The model under review builds one solid part; all positions refer to its coordinate system, in mm. A direction names the side the tool comes from. Round coordinates to 2 decimals unless told otherwise and drop trailing zeros. Loops run counter-clockwise (first coordinate to the right, second up) from the corner with the lowest first, then second, coordinate; pieces in that order, holes last. Notation, with made-up numbers: (-17.5, 56) - (29.5, 56) arc R33 ccw to (29.5, 89) - close; hole circle Ø2 at (-30.75, 75). An arc over 180 degrees is marked (long way). Answer as CSV lines item,"result".
from build123d import *

# Parameters (mm, degrees)
SKETCH_1_R          = 15
EXTRUDE_1_DEPTH     = 2.8
EXTRUDE_2_DEPTH     = 5.4
SKETCH_3_R          = 13.05
EXTRUDE_3_DEPTH     = 7
SKETCH_4_R          = 9.5
CUT_EXTRUDE_1_DEPTH = 13


with BuildPart() as part:
    # 草图1 → 凸台-拉伸1 (new body)
    with BuildSketch(Plane.XY):
        Circle(SKETCH_1_R)
    extrude(amount=EXTRUDE_1_DEPTH)

    # 草图2 → 凸台-拉伸2 (add)
    with BuildSketch(Plane(origin=(0, 0, 0), x_dir=(-1, 0, 0), z_dir=(0, 0, -1))):
        Polygon((6.062177826, -10.5), (12.124355653, 0), (6.062177826, 10.5), (-6.062177826, 10.5), (-12.124355653, 0), (-6.062177826, -10.5), align=None)
    extrude(amount=EXTRUDE_2_DEPTH)

    # 草图3 → 凸台-拉伸3 (add)
    with BuildSketch(Plane.XY.offset(2.8)):
        Circle(SKETCH_3_R)
    extrude(amount=EXTRUDE_3_DEPTH)

    # 草图4 → 切除-拉伸1 (cut)
    with BuildSketch(Plane.XY.offset(9.8)):
        Circle(SKETCH_4_R)
    extrude(amount=-CUT_EXTRUDE_1_DEPTH, mode=Mode.SUBTRACT)


solid = part.part
1. Clearance check with flat-ended pins moving along their axes: pin 1 (2.5 mm diameter, centred on x = -2, z = -3.5, fed in from -Y); pin 2 (6 mm diameter, centred on y = 6.5, z = 0.5, fed in from +X); pin 3 (3 mm diameter, centred on y = 10.5, z = -0.5, fed in from -X). State where each tip first meets the part, or that it passes through.
Numbers:
pin 1,"stops at y = -10.5"
pin 2,"stops at x = 14.59"
pin 3,"stops at x = -11.94"
2. Take a section at D-D (z = -4.25). State the section outline as (x, y) points.
Numbers:
outline,"(-12.12, 0) - (-6.06, -10.5) - (6.06, -10.5) - (12.12, 0) - (6.06, 10.5) - (-6.06, 10.5) - close"
3. Tool access review of faces 1 (the face through (-9.136, 5.176, -2.662)), 2 (the face through (0, -11, 0)), 3 (the face through (-1.2, -13.3, 2.8)): name each direction out of +Z, -Z, +X, -X, +Y, -Y from which nothing blocks a thin tool from reaching the whole face with its end or side.
Numbers:
face 1,"-Z, -X, +Y"
face 2,"-Z"
face 3,"+Z"
4. Take a section at C-C (y = 12). State the section outline as (x, z) points, plus the area to 3 significant figures.
Numbers:
outline,"(-9, 0) - (9, 0) - (9, 2.8) - (5.13, 2.8) - (5.13, 9.8) - (-5.13, 9.8) - (-5.13, 2.8) - (-9, 2.8) - close"
area,"122 mm²"
5. Take a section at A-A (z = -2.5). State the section outline as (x, y) points, plus the area to 3 significant figures.
Numbers:
outline,"(-12.12, 0) - (-6.06, -10.5) - (6.06, -10.5) - (12.12, 0) - (6.06, 10.5) - (-6.06, 10.5) - close; hole circle Ø19 at (0, 0)"
area,"98.4 mm²"
6. Wall thickness on probe 1 along Y at (x, z) = (0.25, -1); probe 2 along Y at (x, z) = (0, 1); probe 3 along X at (y, z) = (7.5, -3): over which ranges is each line inside the solid? List them lowest first.
Numbers:
probe 1,"y = -10.5 to -9.5, 9.5 to 10.5"
probe 2,"y = -15 to -9.5, 9.5 to 15"
probe 3,"x = -7.79 to -5.83, 5.83 to 7.79"
7. Draft analysis for pull direction X (two halves, no side actions). For faces 4 (the face through (4.38, -8.43, 3.39)), 5 (the face through (0, 0, -3.2)), 6 (the face through (-9.051, -5.324, -2.662)), 7 (the face through (1, -10, 9.8)), state which applies: +X half, -X half, draft (parallel to the pull), parting line (faces both ways), or undercut.
Numbers:
face 4,"undercut"
face 5,"undercut"
face 6,"-X half"
face 7,"draft"
8. Take a section at B-B (x = 0). State the section outline as (y, z) points, plus the area to 3 significant figures.
Numbers:
outline,"(-15, 0) - (-10.5, 0) - (-10.5, -5.4) - (10.5, -5.4) - (10.5, 0) - (15, 0) - (15, 2.8) - (13.05, 2.8) - (13.05, 9.8) - (9.5, 9.8) - (9.5, -3.2) - (-9.5, -3.2) - (-9.5, 9.8) - (-13.05, 9.8) - (-13.05, 2.8) - (-15, 2.8) - close"
area,"133 mm²"
